Check sheet for the drawn part. Datum: minimum x, y, z corner. Units: mm. Round coordinates to 2 decimals unless told otherwise and drop trailing zeros. Order: outer loops, then holes, each group sorted by start corner. A loop starts at its lowest first (then second) coordinate and runs counter-clockwise, first axis right, second up.
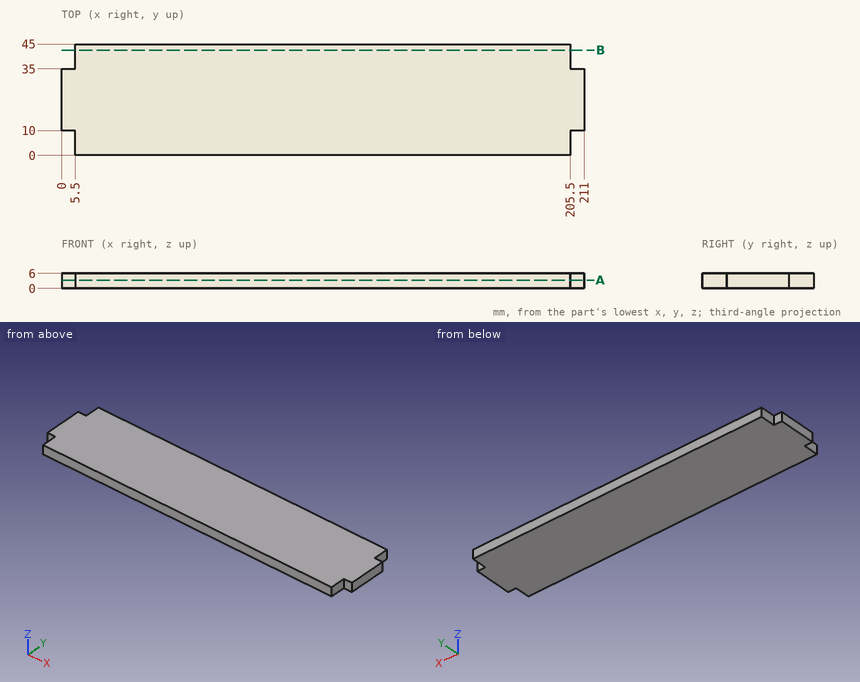
1) Sectioned sample at A-A on z = 3.3. Record the cut outline in (x, y).
2) Gauge pin test, flat ends, axial feed: pin 1 (3 mm diameter, centred on y = 3, z = 3.5, fed in from -X); pin 2 (3 mm diameter, centred on y = 40, z = 2, fed in from +X); pin 3 (3 mm diameter, centred on x = 2, z = 3.5, fed in from -Y). Record the tip position at first contact, or that the pin passes through.
3) Scan line: line 1 (X direction, y = 9.5, z = 5.6). Record every from-to range of solid material in increasing order.
4) Sectioned sample at B-B on y = 42.5. Record the cut outline in (x, z).
Values found:
1. outline: (0, 10) - (5.5, 10) - (5.5, 0) - (205.5, 0) - (205.5, 10) - (211, 10) - (211, 35) - (205.5, 35) - (205.5, 45) - (5.5, 45) - (5.5, 35) - (0, 35) - close
2. pin 1: stops at x = 5.5
2. pin 2: stops at x = 205.5
2. pin 3: stops at y = 10
3. line 1: x = 5.5 to 205.5
4. outline: (5.5, 0) - (205.5, 0) - (205.5, 6) - (5.5, 6) - close
